Source: CAD feature listing. Evaluate the final solid. Frame: model axes, mm. A direction names the side the tool comes from. Give positions to 0.01 mm unless a question says otherwise; leave off trailing zeros. Order: outer loops, then holes, each group sorted by start corner. A loop starts at its lowest first (then second) coordinate and runs counter-clockwise, first axis right, second up.
from build123d import *

# Parameters (mm, degrees)
BASE_PLATE_DEPTH          = 8
MOUNTING_HOLES_SKETCH_R   = 8
MOUNTING_HOLES_2X_DEPTH   = 8
UPRIGHT_DEPTH             = 32
SUPPORT_RIB_REACH         = 79.589
SUPPORT_RIB_SKETCH_WALL_W = 198.408374186
SUPPORT_RIB_SKETCH_WALL_H = 12


with BuildPart() as part:
    # Base Plate Sketch → Base Plate (new body)
    with BuildSketch(Plane(origin=(0, 0, 0), x_dir=(1, 0, 0), z_dir=(0, 1, 0))):
        with BuildLine():
            Line((-46, 18), (46, 18))
            ThreePointArc((46, 18), (64, 0), (46, -18))
            Line((46, -18), (-46, -18))
            ThreePointArc((-46, -18), (-64, 0), (-46, 18))
        make_face()
    extrude(amount=BASE_PLATE_DEPTH)

    # Mounting Holes Sketch → Mounting Holes 2x (cut)
    with BuildSketch(Plane(origin=(0, 8, 0), x_dir=(1, 0, 0), z_dir=(0, 1, 0))):
        with Locations(Location((-46, 0, 0), (0, 0, 270))):
            Circle(MOUNTING_HOLES_SKETCH_R)
        with Locations(Location((46, 0, 0), (0, 0, 270))):
            Circle(MOUNTING_HOLES_SKETCH_R)
    extrude(amount=-MOUNTING_HOLES_2X_DEPTH, mode=Mode.SUBTRACT)

    # Upright Sketch → Upright (add)
    with BuildSketch(Plane(origin=(0, 8, 0), x_dir=(1, 0, 0), z_dir=(0, 1, 0))):
        Polygon((0, 18), (-20, 18), (-20, 8), (20, 8), (20, 18), align=None)
    extrude(amount=UPRIGHT_DEPTH)

    # Support Rib Sketch wall → Support Rib (add, up to next)
    with BuildSketch(Plane(origin=(0, 24, 5), x_dir=(0, -0.776114000116, 0.630592625094), z_dir=(0, -0.630592625094, -0.776114000116)), mode=Mode.PRIVATE) as support_rib_sk1:
        Rectangle(SUPPORT_RIB_SKETCH_WALL_W, SUPPORT_RIB_SKETCH_WALL_H)
    support_rib_tool1 = extrude(support_rib_sk1.sketch, amount=SUPPORT_RIB_REACH, mode=Mode.PRIVATE) - part.part
    add(support_rib_tool1.solids().sort_by_distance((0, 24, 5))[0])


solid = part.part
(1) Section B-B, the plane z = 0. Return loops of the section in (x, y).
(2) Line query: line 1 along X through (y, z) = (1.5, 0); line 2 along X through (y, z) = (5, 3.5); line 3 along Y through (x, z) = (-47, 8). Output: solid intervals per line, ascending.
(3) Section C-C, the plane y = 4. Return loops of the section in (x, z).
(4) Access query for faces 1 (the flat face through (-13, 24, -8)), 2 (the flat face through (20, 24, -13)), 3 (the flat face through (6, 19, -1)), 4 (the flat face through (1, 0, 0)), 5 (the flat face through (-20, 24, -13)). Directions: +Z, -Z, +X, -X, +Y, -Y. A direction counts if a zero-diameter tool reaches every point of the face in a straight line with its end or side. Return the directions, or none.
(5) Draft query along Z for faces 6 (the flat face through (-6, 19, -1)), 7 (the cylindrical face through (-38.068, 4.056, -1.041)), 8 (the cylindrical face through (-64, 4, 0)). Return one class per face: +Z half, -Z half, draft (parallel to the pull), parting line (faces both ways), or undercut.
(6) Pin query (flat end, axial travel): pin 1 Ø6 at (x, z) = (3.5, 10.5) entering from +Y; pin 2 Ø18 at (x, z) = (-24.5, 6) entering from +Y; pin 3 Ø1 at (y, z) = (5, 6.5) entering from -X. Return the tip coordinate at first contact, or that it passes through.
(7) Section A-A, the plane x = -52. Return loops of the section in (y, z).
(8) Section D-D, the plane x = -17.5. Return loops of the section in (y, z), plus the area to 3 significant figures.
Checks:
1. outline: (-64, 0) - (-54, 0) - (-54, 8) - (-64, 8) - close; (-38, 0) - (38, 0) - (38, 8) - (6, 8) - (6, 30.15) - (-6, 30.15) - (-6, 8) - (-38, 8) - close; (54, 0) - (64, 0) - (64, 8) - (54, 8) - close
2. line 1: x = -64 to -54, -38 to 38, 54 to 64
2. line 2: x = -63.66 to -53.19, -38.81 to 38.81, 53.19 to 63.66
2. line 3: y = 0 to 8
3. outline: (-46, -18) - (46, -18) arc R18 ccw to (46, 18) - (-46, 18) arc R18 ccw to start; hole circle Ø16 at (-46, 0); hole circle Ø16 at (46, 0)
4. face 1: +Z, -X, +Y
4. face 2: +Z, -Z, +X, +Y
4. face 3: +Z, +X, +Y
4. face 4: +Z, -Z, +X, -X, -Y
4. face 5: +Z, -Z, -X, +Y
5. face 6: draft
5. face 7: undercut
5. face 8: parting line
6. pin 1: stops at y = 20.92
6. pin 2: stops at y = 8
6. pin 3: stops at x = -62.97
7. outline: (0, -16.97) - (8, -16.97) - (8, -5.29) - (0, -5.29) - close; (0, 5.29) - (8, 5.29) - (8, 16.97) - (0, 16.97) - close
8. outline: (0, -18) - (40, -18) - (40, -8) - (8, -8) - (8, 18) - (0, 18) - close
8. area: 608 mm2
